The listing builds one solid part. Answer for the finished solid, in the listing's coordinates (mm). Face numbers are marked on the shaded views. A direction names the side the tool comes from. Give positions to 0.01 mm unless a question says otherwise; leave off trailing zeros. Order: outer loops, then holes, each group sorted by start corner. A loop starts at its lowest first (then second) coordinate and runs counter-clockwise, first axis right, second up. Notation, with made-up numbers: (-33, 40) - (-28, 40) arc R18 cw to (-28, 72) - close; hole circle Ø10 at (-31.75, 69.5). An arc over 180 degrees is marked (long way). Answer as CSV lines item,"result". Start each with the question number.
1. Section A-A on x = 0 is taken. Give the vertices of the cut face in (y, z).
2. Section B-B on z = 0 is taken. Give the vertices of the cut face in (x, y).
3. Section C-C on x = -1.6 is taken. Give the vertices of the cut face in (y, z).
4. Which of the six approach directions +Z, -Z, +X, -X, +Y, -Y give full straight-line access (tool end or side, diameter ignored) to the marked faces 1 and 2?
5. Consider line 1 along X through (y, z) = (7.75, 0); line 2 along X through (y, z) = (2.75, 0.8); line 3 along Z through (x, y) = (0.2, 15). Determine where each line is inside the solid, lowest interval first. Write a range as [from, to].
6. Section D-D on y = 5 is taken. Give the vertices of the cut face in (x, z), and give its area (3 significant figures).
7. Flat-ended cylindrical pins translate along their axes: pin 1 (1.5 mm diameter, centred on y = 12.5, z = 1, fed in from -X); pin 2 (1.5 mm diameter, centred on y = 12.5, z = 1, fed in from +X). Find the tip coordinate at first contact, or state that the pin passes through.
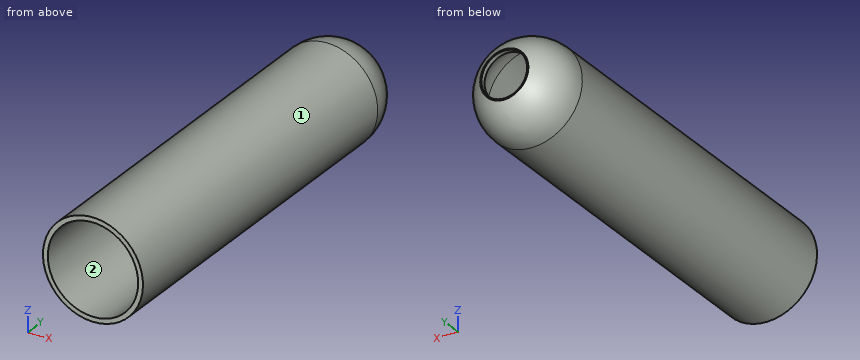
from build123d import *


with BuildPart() as part:
    # Sketch1 → Revolve1 (revolve)
    with BuildSketch(Plane.XY, mode=Mode.PRIVATE) as revolve1_sk:
        with BuildLine():
            Line((-2.18, 0), (-2.18, 16))
            ThreePointArc((-2.18, 16), (-1.876352845, 17.109819805), (-1.05, 17.910471146))
            Line((-1.05, 17.910471146), (-0.994634547, 17.910471146))
            Line((-0.994634547, 17.910471146), (-0.994634547, 17.700471146))
            ThreePointArc((-0.994634547, 17.700471146), (-1.708849036, 16.980170889), (-1.97, 16))
            Line((-1.97, 16), (-1.97, 0))
            Line((-1.97, 0), (-2.18, 0))
        make_face()
    revolve(revolve1_sk.sketch.rotate(Axis((0, 0, 0), (0, 1, 0)), 270), axis=Axis((0, 0, 0), (0, 1, 0)))


solid = part.part
Checks:
1,outline,"(0, -2.18) - (16, -2.18) arc R2.18 ccw to (17.91, -1.05) - (17.91, -0.99) - (17.7, -0.99) arc R1.97 cw to (16, -1.97) - (0, -1.97) - close; (0, 1.97) - (16, 1.97) arc R1.97 cw to (17.7, 0.99) - (17.91, 0.99) - (17.91, 1.05) arc R2.18 ccw to (16, 2.18) - (0, 2.18) - close"
2,outline,"(-2.18, 0) - (-1.97, 0) - (-1.97, 16) arc R1.97 cw to (-0.99, 17.7) - (-0.99, 17.91) - (-1.05, 17.91) arc R2.18 ccw to (-2.18, 16) - close; (0.99, 17.7) arc R1.97 cw to (1.97, 16) - (1.97, 0) - (2.18, 0) - (2.18, 16) arc R2.18 ccw to (1.05, 17.91) - (0.99, 17.91) - close"
3,outline,"(0, -1.48) - (16, -1.48) arc R1.48 ccw to (16, 1.48) - (0, 1.48) - (0, 1.15) - (16, 1.15) arc R1.15 cw to (16, -1.15) - (0, -1.15) - close"
4,face 1,"+Y, -Y"
4,face 2,"-Y"
5,line 1,"x = [-2.18, -1.97], [1.97, 2.18]"
5,line 2,"x = [-2.03, -1.8], [1.8, 2.03]"
5,line 3,"z = [-2.17, -1.96], [1.96, 2.17]"
6,outline,"circle Ø4.36 at (0, 0); hole circle Ø3.94 at (0, 0)"
6,area,"2.74 mm²"
7,pin 1,"stops at x = -2.17"
7,pin 2,"stops at x = 2.17"
